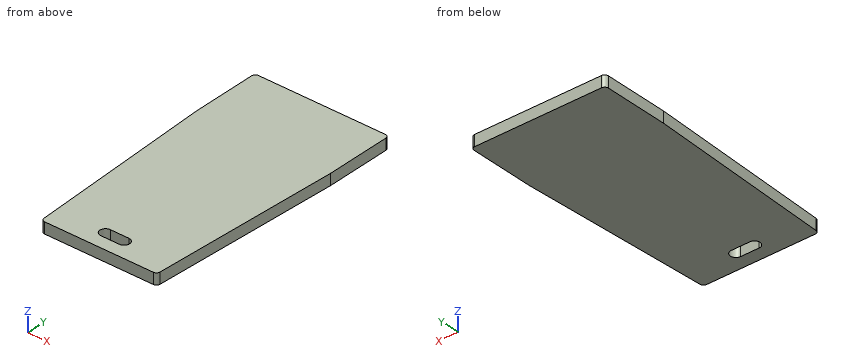
```python
from build123d import *

# Parameters (mm, degrees)
BOSS_EXTRUDE1_DEPTH = 9.525


with BuildPart() as part:
    # Sketch1 → Boss-Extrude1 (new, symmetric)
    with BuildSketch(Plane.XY):
        with BuildLine():
            Line((108.65, 415.8), (-108.65, 415.8))
            ThreePointArc((-108.65, 415.8), (-113.140128061, 413.940128061), (-115, 409.45))
            Line((-115, 409.45), (-115, 298.68))
            Line((-115, 298.68), (-99.351565081, -25.705969286))
            ThreePointArc((-99.351565081, -25.705969286), (-97.389556909, -29.997031921), (-93.008940798, -31.75))
            Line((-93.008940798, -31.75), (93.008940798, -31.75))
            ThreePointArc((93.008940798, -31.75), (97.389556909, -29.997031921), (99.351565081, -25.705969286))
            Line((99.351565081, -25.705969286), (115, 298.68))
            Line((115, 298.68), (115, 409.45))
            ThreePointArc((115, 409.45), (113.140128061, 413.940128061), (108.65, 415.8))
        make_face()
        with BuildLine():
            Line((-15.875, 9.525), (15.875, 9.525))
            ThreePointArc((15.875, 9.525), (25.4, 0), (15.875, -9.525))
            Line((15.875, -9.525), (-15.875, -9.525))
            ThreePointArc((-15.875, -9.525), (-25.4, 0), (-15.875, 9.525))
        make_face(mode=Mode.SUBTRACT)
    extrude(amount=BOSS_EXTRUDE1_DEPTH, both=True)


solid = part.part
```
Build history of the part. All positions in model axes, mm. Round coordinates to 2 decimals unless told otherwise and drop trailing zeros. Loops run counter-clockwise (first coordinate to the right, second up) from the corner with the lowest first, then second, coordinate; pieces in that order, holes last.
Item 1: Drill centre lines: line 1 along Y through (x, z) = (6.5, 6.25) (3 decimals); line 2 along Y through (x, z) = (19, -4.75); line 3 along X through (y, z) = (217, -6.25). Where is each one in solid material? Low to high.
Item 2: Saw through at B-B (y = 0). List the corners of the cut face in (x, z) (3 decimals), then the cut area to 3 significant figures.
Item 3: Saw through at A-A (z = 3.75). List the corners of the cut face in (x, y) (3 decimals).
Item 4: Saw through at D-D (y = 118). List the corners of the cut face in (x, z) (3 decimals), then the cut area to 3 significant figures.
Item 5: Saw through at C-C (y = 230). List the corners of the cut face in (x, z) (3 decimals), then the cut area to 3 significant figures.
Item 6: Pin check, flat tips, straight feed: P1, Ø4, axis at y = 44, z = -4.5, coming from the -X side; P2, Ø8, axis at y = 80.5, z = -3.5, coming from the -X side; P3, Ø8, axis at y = 217.5, z = -7, coming from the -X side. Stop position of each tip, or through.
Worked answers:
1. line 1: y = -31.75 to -9.525, 9.525 to 415.8
1. line 2: y = -31.75 to -9, 9 to 415.8
1. line 3: x = -111.06 to 111.06
2. outline: (-100.592, -9.525) - (-25.4, -9.525) - (-25.4, 9.525) - (-100.592, 9.525) - close; (25.4, -9.525) - (100.592, -9.525) - (100.592, 9.525) - (25.4, 9.525) - close
2. area: 2,860 mm2
3. outline: (-115, 298.68) - (-99.352, -25.706) arc R6.35 ccw to (-93.009, -31.75) - (93.009, -31.75) arc R6.35 ccw to (99.352, -25.706) - (115, 298.68) - (115, 409.45) arc R6.35 ccw to (108.65, 415.8) - (-108.65, 415.8) arc R6.35 ccw to (-115, 409.45) - close; hole (-15.875, -9.525) - (15.875, -9.525) arc R9.525 ccw to (15.875, 9.525) - (-15.875, 9.525) arc R9.525 ccw to start
4. outline: (-106.284, -9.525) - (106.284, -9.525) - (106.284, 9.525) - (-106.284, 9.525) - close
4. area: 4,050 mm2
5. outline: (-111.687, -9.525) - (111.687, -9.525) - (111.687, 9.525) - (-111.687, 9.525) - close
5. area: 4,260 mm2
6. P1: stops at x = -102.81
6. P2: stops at x = -104.67
6. P3: stops at x = -111.28
